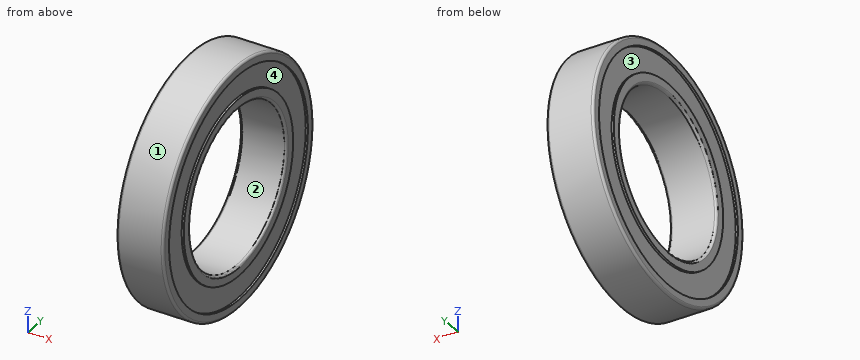
```python
from build123d import *

# Parameters (mm, degrees)
FILLET1_R = 0.6
FILLET2_R = 0.6


with BuildPart() as part:
    # Sketch1 → Revolve1 (revolve)
    with BuildSketch(Plane.XY, mode=Mode.PRIVATE) as revolve1_sk:
        Polygon((0, 20), (12, 20), (12, 22.6), (11.45, 22.6), (11.45, 28.7), (12, 28.7), (12, 31), (0, 31), (0, 28.7), (0.55, 28.7), (0.55, 22.6), (0, 22.6), align=None)
    revolve(revolve1_sk.sketch.rotate(Axis((0, 0, 0), (1, 0, 0)), 180), axis=Axis((0, 0, 0), (1, 0, 0)))

    # Fillet1
    fillet1_edges = [part.edges().sort_by_distance(p)[0] for p in [
        (0, 31, 0),
        (12, 31, 0),
    ]]
    fillet(fillet1_edges, radius=FILLET1_R)

    # Fillet2
    fillet2_edges = [part.edges().sort_by_distance(p)[0] for p in [
        (12, 20, 0),
        (0, 20, 0),
    ]]
    fillet(fillet2_edges, radius=FILLET2_R)


solid = part.part
```
The model under review builds one solid part; all positions refer to its coordinate system, in mm. Face numbers are marked on the shaded views. A direction names the side the tool comes from. Round coordinates to 2 decimals unless told otherwise and drop trailing zeros. Order: outer loops, then holes, each group sorted by start corner. A loop starts at its lowest first (then second) coordinate and runs counter-clockwise, first axis right, second up.
Item 1: Draft analysis for pull direction Y (two halves, no side actions). For the marked faces 1 and 2, state which applies: released by +Y, released by -Y, zero draft, split by the parting line, or undercut.
Working result:
face 1: split by the parting line
face 2: undercut
Item 2: Machinability: for the marked faces 3 and 4, which of the approach directions +Z, -Z, +X, -X, +Y, -Y give a long, thin tool a straight path to every point of the face, cutting with its end or side? Answer none if there is none.
Working result:
face 3: -X
face 4: +X
Item 3: For pin 1 (4 mm diameter, centred on x = 8, y = -24, fed in from +Z); pin 2 (1.5 mm diameter, centred on x = 5, z = 8.5, fed in from +Y); pin 3 (4 mm diameter, centred on x = 7, y = 10, fed in from -Z); pin 4 (24 mm diameter, centred on y = 0, z = 0, fed in from -X), all flat-tipped, find the tip position at first contact; note any pin that passes through.
Working result:
pin 1: stops at z = 21.84
pin 2: stops at y = 30.02
pin 3: stops at z = -29.95
pin 4: passes through
Item 4: Add section C-C, the plane x = 7.5. State the section outline as (y, z) points.
Working result:
outline: circle Ø62 at (0, 0); hole circle Ø40 at (0, 0)
Item 5: To check wall thickness, follow probe 1 along Z at (x, y) = (0.2, 0); probe 2 along Z at (x, y) = (8.75, 0); probe 3 along Z at (x, y) = (0.4, 0). State the ranges of each line that lie inside material, in increasing order.
Working result:
probe 1: z = -30.85 to -28.7, -22.6 to -20.15, 20.15 to 22.6, 28.7 to 30.85
probe 2: z = -31 to -20, 20 to 31
probe 3: z = -30.97 to -28.7, -22.6 to -20.03, 20.03 to 22.6, 28.7 to 30.97
